```python
from build123d import *

# Parameters (mm, degrees)
BOSS_EXTRUDE1_DEPTH = 5
SKETCH2_R           = 7.5
BOSS_EXTRUDE2_DEPTH = 10
BOSS_EXTRUDE7_START = 10
SKETCH9_R           = 7.5
BOSS_EXTRUDE7_DEPTH = 10
SKETCH3_W           = 9.261773254
SKETCH3_H           = 43.8
BOSS_EXTRUDE3_DEPTH = 4
SKETCH4_W           = 9.261773254
SKETCH4_H           = 11.9
BOSS_EXTRUDE4_DEPTH = 5.03
SKETCH5_R           = 7.423962758
BOSS_EXTRUDE5_DEPTH = 2
BOSS_EXTRUDE6_DEPTH = 3
SKETCH7_R           = 2.850666807
CUT_EXTRUDE1_DEPTH  = 0.1
CUT_EXTRUDE2_DEPTH  = 1


with BuildPart() as part:
    # Sketch1 → Boss-Extrude1 (new body)
    with BuildSketch(Plane(origin=(0, 0, 0), x_dir=(1, 0, 0), z_dir=(0, 1, 0))):
        Polygon((5.773502692, 10), (-5.773502692, 10), (-11.547005384, 0), (-5.773502692, -10), (5.773502692, -10), (11.547005384, 0), align=None)
    extrude(amount=BOSS_EXTRUDE1_DEPTH)

    # Sketch2 → Boss-Extrude2 (add)
    with BuildSketch(Plane.XZ):
        with Locations(Location((0, 0, 0), (0, 0, 270))):
            Circle(SKETCH2_R)
    extrude(amount=BOSS_EXTRUDE2_DEPTH)

    # Sketch9 → Boss-Extrude7 (add)
    with BuildSketch(Plane(origin=(0, 5, 0), x_dir=(1, 0, 0), z_dir=(0, 1, 0)).offset(BOSS_EXTRUDE7_START)):
        with Locations(Location((0, 0, 0), (0, 0, 90))):
            Circle(SKETCH9_R)
    extrude(amount=-BOSS_EXTRUDE7_DEPTH)

    # Sketch3 → Boss-Extrude3 (add)
    with BuildSketch(Plane(origin=(0, 15, 0), x_dir=(1, 0, 0), z_dir=(0, 1, 0))):
        Rectangle(SKETCH3_W, SKETCH3_H)
    extrude(amount=BOSS_EXTRUDE3_DEPTH)

    # Sketch4 → Boss-Extrude4 (add)
    with BuildSketch(Plane(origin=(0, 19, 0), x_dir=(1, 0, 0), z_dir=(0, 1, 0))):
        with Locations((0, 15.95)):
            Rectangle(SKETCH4_W, SKETCH4_H)
        with Locations((0, -15.95)):
            Rectangle(SKETCH4_W, SKETCH4_H)
    extrude(amount=BOSS_EXTRUDE4_DEPTH)

    # Sketch5 → Boss-Extrude5 (add)
    with BuildSketch(Plane(origin=(0, 19, 0), x_dir=(1, 0, 0), z_dir=(0, 1, 0))):
        with Locations(Location((0, 0, 0), (0, 0, 51.407625877))):
            Circle(SKETCH5_R)
    extrude(amount=BOSS_EXTRUDE5_DEPTH)

    # Sketch6 → Boss-Extrude6 (add)
    with BuildSketch(Plane(origin=(0, 21, 0), x_dir=(1, 0, 0), z_dir=(0, 1, 0))):
        Polygon((0, 4.871086868), (-4.218484972, 2.435543434), (-4.218484972, -2.435543434), (0, -4.871086868), (4.218484972, -2.435543434), (4.218484972, 2.435543434), align=None)
    extrude(amount=BOSS_EXTRUDE6_DEPTH)

    # Sketch7 → Cut-Extrude1 (cut)
    with BuildSketch(Plane(origin=(0, 24.03, 0), x_dir=(1, 0, 0), z_dir=(0, 1, 0))):
        with Locations(Location((0, 14.250511049, 0), (0, 0, 270))):
            Circle(SKETCH7_R)
        with Locations(Location((0, -14.372767949, 0), (0, 0, 270))):
            Circle(SKETCH7_R)
    extrude(amount=-CUT_EXTRUDE1_DEPTH, mode=Mode.SUBTRACT)

    # Sketch8 → Cut-Extrude2 (cut)
    with BuildSketch(Plane(origin=(0, 23.93, 0), x_dir=(1, 0, 0), z_dir=(0, 1, 0))):
        Polygon((-1.343066927, 11.719300444), (0.804329856, 17.000767289), (1.330666503, 16.786763555), (-0.81673028, 11.505296711), align=None)
        Polygon((-1.076876675, -17.027451515), (0.531783037, -11.557769723), (1.076876675, -11.718084383), (-0.531783037, -17.187766175), align=None)
    extrude(amount=-CUT_EXTRUDE2_DEPTH, mode=Mode.SUBTRACT)


solid = part.part
```
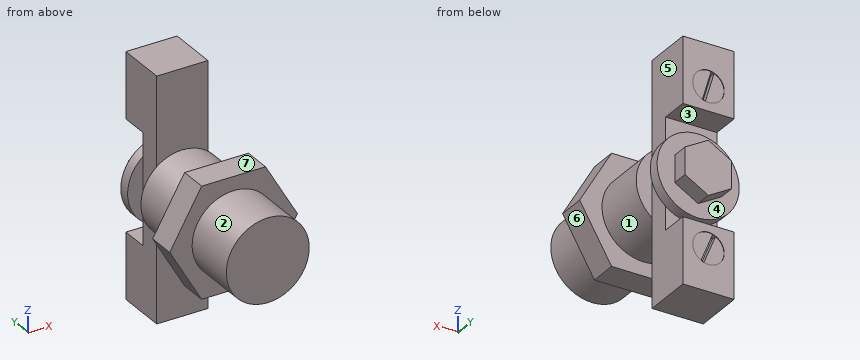
The model under review builds one solid part; all positions refer to its coordinate system, in mm. Face numbers are marked on the shaded views. A direction names the side the tool comes from. Round coordinates to 2 decimals unless told otherwise and drop trailing zeros. Write each loop counter-clockwise with the first axis right and the second up, starting at its lowest first coordinate (ties: lowest second). Pieces come first, ordered by that corner, then holes.
(1) Machinability: for the marked faces 1, 2 and 3, which of the approach directions +Z, -Z, +X, -X, +Y, -Y give a long, thin tool a straight path to every point of the face, cutting with its end or side? Answer none if there is none.
(2) We need section B-B on y = -2. Give the boundary of the cut face in (x, z), and give its area (3 significant figures).
(3) We need section C-C on z = 11. Give the boundary of the cut face in (x, y).
(4) We need section D-D on x = 10.25. Give the boundary of the cut face in (y, z), and give its area (3 significant figures).
(5) Wall thickness on L1, parallel to Z at x = -1.25, y = 22; L2, parallel to Z at x = 4.25, y = 1.5; L3, parallel to Y at x = 8.5, z = 4: over which ranges is each line inside the solid? List them lowest first.
(6) Mouldability with a two-part tool opening along Z and no side actions: class the marked faces 4, 5, 6 and 7 as +Z half, -Z half, draft (parallel to the pull), parting line (faces both ways), or undercut.
(7) We need section A-A on z = -8. Give the boundary of the cut face in (x, y), and give its area (3 significant figures).
(8) Insertion check: pin 1 (2 mm diameter, centred on x = -1, y = -5, fed in from -Z); pin 2 (4 mm diameter, centred on y = 18.5, z = -1.5, fed in from +X); pin 3 (2.5 mm diameter, centred on x = 1, y = 2, fed in from +Z). Each pin has a flat end and moves straight along its axis. Give the tip position at first contact, or say it passes through.
Findings below:
1. face 1: none
1. face 2: -Y
1. face 3: +X, -X, +Y
2. outline: circle Ø15 at (0, 0)
2. area: 177 mm2
3. outline: (-4.63, 15) - (4.63, 15) - (4.63, 24.03) - (-4.63, 24.03) - close
4. outline: (0, -2.25) - (5, -2.25) - (5, 2.25) - (0, 2.25) - close
4. area: 22.5 mm2
5. L1: z = -21.9 to -10, -4.15 to 4.15, 10 to 21.9
5. L2: z = -10 to 10
5. L3: y = 0 to 5
6. face 4: undercut
6. face 5: draft
6. face 6: -Z half
6. face 7: +Z half
7. outline: (-6.93, 0) - (6.93, 0) - (6.93, 5) - (-6.93, 5) - close; (-4.63, 15) - (4.63, 15) - (4.63, 19) - (-4.63, 19) - close
7. area: 106 mm2
8. pin 1: stops at z = -7.5
8. pin 2: stops at x = 7.42
8. pin 3: stops at z = 10
